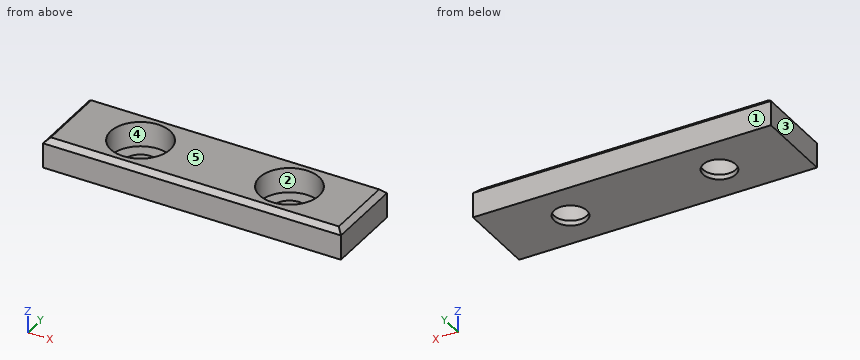
from build123d import *

# Parameters (mm, degrees)
SKETCH1_W          = 60
SKETCH1_H          = 16
BASE_EXTRUDE_DEPTH = 6
SKETCH2_R          = 3.3
CUT_EXTRUDE1_DEPTH = 49.840144417
SKETCH3_R          = 6
CUT_EXTRUDE2_DEPTH = 5
LPATTERN1_COUNT    = 2
LPATTERN1_PITCH    = 30
CHAMFER1_SIZE      = 1


with BuildPart() as part:
    # Sketch1 → Base-Extrude (new body)
    with BuildSketch(Plane.XY):
        with Locations((17.371751412, -2.260451977)):
            Rectangle(SKETCH1_W, SKETCH1_H)
    extrude(amount=BASE_EXTRUDE_DEPTH)

    # Sketch2 → Cut-Extrude1 (cut, through all)
    with BuildSketch(Plane.XY.offset(6)):
        with Locations((2.371751412, -2.260451977)):
            Circle(SKETCH2_R)
    cut_extrude1 = extrude(amount=-CUT_EXTRUDE1_DEPTH, mode=Mode.SUBTRACT)

    # Sketch3 → Cut-Extrude2 (cut)
    with BuildSketch(Plane.XY.offset(6)):
        with Locations((2.371751412, -2.260451977)):
            Circle(SKETCH3_R)
    cut_extrude2 = extrude(amount=-CUT_EXTRUDE2_DEPTH, mode=Mode.SUBTRACT)

    # LPattern1: Cut-Extrude1, Cut-Extrude2 ×2
    with Locations(*[(i * LPATTERN1_PITCH, 0, 0) for i in range(1, LPATTERN1_COUNT)]):
        add(cut_extrude1, mode=Mode.SUBTRACT)
        add(cut_extrude2, mode=Mode.SUBTRACT)

    # Chamfer1
    chamfer1_edges = [part.edges().sort_by_distance(p)[0] for p in [
        (47.371751412, -2.260451977, 6),
        (17.371751412, 5.739548023, 6),
        (-12.628248588, -2.260451977, 6),
        (17.371751412, -10.260451977, 6),
    ]]
    chamfer(chamfer1_edges, length=CHAMFER1_SIZE)


solid = part.part
Check sheet for the modelled part. Datum: model origin and axes. Units: mm. Face numbers are marked on the shaded views. A direction names the side the tool comes from. Give positions to 0.01 mm unless a question says otherwise; leave off trailing zeros. Loops run counter-clockwise (first coordinate to the right, second up) from the corner with the lowest first, then second, coordinate; pieces in that order, holes last. Notation, with made-up numbers: M 79.5,-19.75 L 131.5,-19.75 A16 ccw 131.5,-4.75 Z; hole C -31,-2 d11. An arc over 180 degrees is marked long. Return JSON: item names as keys, results as strings. Group by question number.
1. Go/stop test with a flat-tipped pin: pin 1 (5.5 mm diameter, centred on x = 32.37, y = -2.26, fed in from -Z). Record where the tip stops, or that it passes through.
2. Cross-section at A-A on y = 0. Record the boundary of the cut face in (x, z).
3. Cross-section at C-C on y = -7.25. Record the boundary of the cut face in (x, z).
4. Mould release check, pull along X, two halves, no side actions. Record for the marked faces 1, 2 and 3: released by +X, released by -X, zero draft, split by the parting line, or undercut.
5. Thickness scan on L1, parallel to X at y = -0.5, z = 4.25; L2, parallel to X at y = 0.5, z = 4.25; L3, parallel to Z at x = 36, y = 0.5. Record the ranges inside material, lowest first.
6. Cross-section at D-D on x = 6.5. Record the boundary of the cut face in (y, z).
7. Tool access check on the marked faces 4 and 5. Record the directions out of +Z, -Z, +X, -X, +Y, -Y that give a thin tool (end or side, any length) a straight path to the whole face; none if there is none.
8. Cross-section at B-B on z = 4. Record the boundary of the cut face in (x, y), plus the area to 3 significant figures.
Return value:
{
 "1": {"pin 1": "through"},
 "2": {"outline": "M -12.63,0 L -0.03,0 L -0.03,1 L -3.19,1 L -3.19,6 L -11.63,6 L -12.63,5 Z; M 4.78,0 L 29.97,0 L 29.97,1 L 26.81,1 L 26.81,6 L 7.93,6 L 7.93,1 L 4.78,1 Z; M 34.78,0 L 47.37,0 L 47.37,5 L 46.37,6 L 37.93,6 L 37.93,1 L 34.78,1 Z"},
 "3": {"outline": "M -12.63,0 L 47.37,0 L 47.37,5 L 46.37,6 L 35.7,6 L 35.7,1 L 29.04,1 L 29.04,6 L 5.7,6 L 5.7,1 L -0.96,1 L -0.96,6 L -11.63,6 L -12.63,5 Z"},
 "4": {"face 1": "zero draft", "face 2": "undercut", "face 3": "released by -X"},
 "5": {"L1": "-12.63 to -3.36, 8.11 to 26.64, 38.11 to 47.37", "L2": "-12.63 to -2.96, 7.7 to 27.04, 37.7 to 47.37", "L3": "0 to 1"},
 "6": {"outline": "M -10.26,0 L 5.74,0 L 5.74,5 L 4.74,6 L 2.09,6 L 2.09,1 L -6.61,1 L -6.61,6 L -9.26,6 L -10.26,5 Z"},
 "7": {"face 4": "+Z", "face 5": "+Z, +X, -X, +Y, -Y"},
 "8": {"outline": "M -12.63,-10.26 L 47.37,-10.26 L 47.37,5.74 L -12.63,5.74 Z; hole C 2.37,-2.26 d12; hole C 32.37,-2.26 d12", "area": "734 mm^2"}
}
